The listing builds one solid part. Answer for the finished solid, in the listing's coordinates (mm). Face numbers are marked on the shaded views. A direction names the side the tool comes from. Give positions to 0.01 mm unless a question says otherwise; leave off trailing zeros. Loops run counter-clockwise (first coordinate to the right, second up) from the corner with the lowest first, then second, coordinate; pieces in that order, holes last. Notation, with made-up numbers: (59.25, 27.5) - (85.25, 27.5) arc R26 ccw to (85.25, 63.5) - close; hole circle Ø6 at (-4, 29). An arc over 180 degrees is marked (long way). Answer as CSV lines item,"result". Start each with the question number.
1) A cutting plane is placed at B-B (x = -0.75). Determine the outline of the cut face in (y, z), and give its area (3 significant figures).
2) A cutting plane is placed at C-C (y = 0). Determine the outline of the cut face in (x, z).
3) A cutting plane is placed at A-A (x = 1.5). Determine the outline of the cut face in (y, z).
4) Find the intervals of material crossed by line 1 along Z through (x, y) = (-0.75, 1.05); line 2 along Y through (x, z) = (0, 0.3); line 3 along Y through (x, z) = (11, 0.15), in increasing order.
5) For a pull along Y with two mould halves and no side action, classify the marked faces 1, 2 and 3 as pulls with the +Y half, pulls with the -Y half, needs draft (parallel to the pull), parting line crosses it, or undercut.
6) Flat-ended cylindrical pins translate along their axes: pin 1 (0.8 mm diameter, centred on x = 0.5, z = 0, fed in from +Y); pin 2 (0.8 mm diameter, centred on x = 9, z = 0, fed in from -Y). Find the tip coordinate at first contact, or state that the pin passes through.
7) A cutting plane is placed at D-D (x = 7.25). Determine the outline of the cut face in (y, z), and give its area (3 significant figures).
8) For the marked faces 4, 5, 6, 7 and 8, determine the directions among +Z, -Z, +X, -X, +Y, -Y from which every point of the face is accessible in a straight line to the end or side of a thin tool.
```python
from build123d import *

# Parameters (mm, degrees)
SALIENTE_EXTRUIR1_DEPTH = 4
SALIENTE_EXTRUIR2_DEPTH = 1.5
CROQUIS3_W              = 15
CROQUIS3_H              = 4
CORTAR_EXTRUIR1_DEPTH   = 52.086410566
CROQUIS4_R              = 1.65
CORTAR_EXTRUIR2_DEPTH   = 54.601779767
FILLET2_R               = 1
SCALE1_SCALE            = 0.3
SKETCH2_R               = 15.04592303
CUT_EXTRUDE3_DEPTH      = 0.4
SKETCH3_R               = 13.988720819
CUT_EXTRUDE4_DEPTH      = 0.4
SKETCH4_W               = 4.5
SKETCH4_H               = 0.1
BOSS_EXTRUDE1_DEPTH     = 1.6
SKETCH5_R               = 0.55
CUT_EXTRUDE5_DEPTH      = 4.4


with BuildPart() as part:
    # Sketch1 → Saliente-Extruir1 (new, symmetric)
    with BuildSketch(Plane.XY):
        with BuildLine():
            Line((-6, 0), (-6, 6))
            Line((-6, 6), (14, 6))
            Line((14, 6), (27.788799976, 17.570176974))
            ThreePointArc((27.788799976, 17.570176974), (36.898130887, 20.772215113), (30.630237093, 13.427389365))
            Line((30.630237093, 13.427389365), (17.60748156, 2.5))
            Line((17.60748156, 2.5), (35.60748156, 2.5))
            ThreePointArc((35.60748156, 2.5), (44.937608579, 0), (35.60748156, -2.5))
            Line((35.60748156, -2.5), (17.60748156, -2.5))
            Line((17.60748156, -2.5), (30.630237093, -13.427389365))
            ThreePointArc((30.630237093, -13.427389365), (36.898130887, -20.772215113), (27.788799976, -17.570176974))
            Line((27.788799976, -17.570176974), (14, -6))
            Line((14, -6), (-6, -6))
            Line((-6, -6), (-6, 0))
        make_face()
    extrude(amount=SALIENTE_EXTRUIR1_DEPTH, both=True)

    # Croquis2 → Saliente-Extruir2 (add, symmetric)
    with BuildSketch(Plane.XY):
        with BuildLine():
            Line((26.884808669, 10.284601755), (14.628097579, 0))
            Line((14.628097579, 0), (26.884808669, -10.284601755))
            ThreePointArc((26.884808669, -10.284601755), (27.660138353, -4.406075759), (31.628097579, 0))
            ThreePointArc((31.628097579, 0), (27.660138353, 4.406075759), (26.884808669, 10.284601755))
        make_face()
    extrude(amount=SALIENTE_EXTRUIR2_DEPTH, both=True)

    # Croquis3 → Cortar-Extruir1 (cut, through all)
    with BuildSketch(Plane.XY.offset(4)):
        with Locations((1.5, 0)):
            Rectangle(CROQUIS3_W, CROQUIS3_H)
    extrude(amount=-CORTAR_EXTRUIR1_DEPTH, mode=Mode.SUBTRACT)

    # Croquis4 → Cortar-Extruir2 (cut, through all)
    with BuildSketch(Plane(origin=(0, 6, 0), x_dir=(1, 0, 0), z_dir=(0, 1, 0))):
        with Locations(Location((-2.5, 0, 0), (0, 0, 180))):
            Circle(CROQUIS4_R)
    extrude(amount=-CORTAR_EXTRUIR2_DEPTH, mode=Mode.SUBTRACT)

    # Fillet2
    fillet2_edges = [part.edges().sort_by_distance(p)[0] for p in [
        (27.034037659, -6.190607199, -1.5),
        (27.034037659, 6.190607199, -1.5),
        (27.034037659, -6.190607199, 1.5),
        (27.034037659, 6.190607199, 1.5),
    ]]
    fillet(fillet2_edges, radius=FILLET2_R)


with BuildPart() as part_1:
    # Scale1: scaled about (0, 0, 0)
    add(part.part.scale(SCALE1_SCALE))

    # Sketch2 → Cut-Extrude3 (cut)
    with BuildSketch(Plane.XY.offset(1.2)):
        Circle(SKETCH2_R)
    extrude(amount=-CUT_EXTRUDE3_DEPTH, mode=Mode.SUBTRACT)

    # Sketch3 → Cut-Extrude4 (cut)
    with BuildSketch(Plane(origin=(0, 0, -1.2), x_dir=(-1, 0, 0), z_dir=(0, 0, -1))):
        Circle(SKETCH3_R)
    extrude(amount=-CUT_EXTRUDE4_DEPTH, mode=Mode.SUBTRACT)

    # Sketch4 → Boss-Extrude1 (add)
    with BuildSketch(Plane.XY.offset(0.8)):
        with Locations((0.45, -0.55)):
            Rectangle(SKETCH4_W, SKETCH4_H)
        with Locations((0.45, 0.55)):
            Rectangle(SKETCH4_W, SKETCH4_H)
    extrude(amount=-BOSS_EXTRUDE1_DEPTH)

    # Sketch5 → Cut-Extrude5 (cut)
    with BuildSketch(Plane.XZ.offset(1.8)):
        with Locations((-0.75, 0)):
            Circle(SKETCH5_R)
    extrude(amount=-CUT_EXTRUDE5_DEPTH, mode=Mode.SUBTRACT)


solid = part_1.part
```
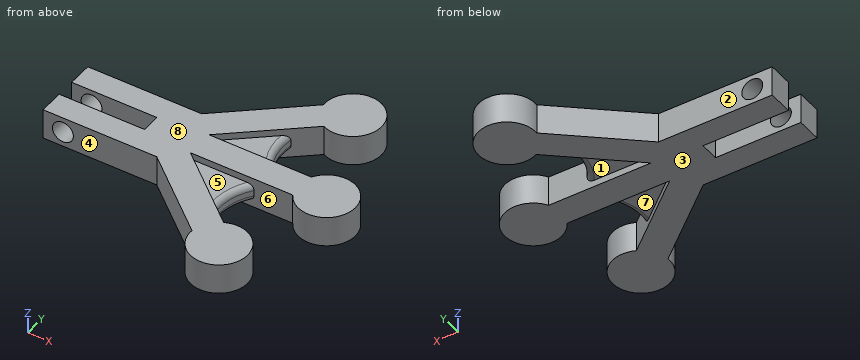
Ans:
1,outline,"(-1.8, -0.8) - (-0.5, -0.8) - (-0.5, -0.55) - (-1.8, -0.55) - close; (-1.8, 0.55) - (-0.5, 0.55) - (-0.5, 0.8) - (-1.8, 0.8) - close; (0.5, -0.8) - (1.8, -0.8) - (1.8, -0.55) - (0.5, -0.55) - close; (0.5, 0.55) - (1.8, 0.55) - (1.8, 0.8) - (0.5, 0.8) - close"
1,area,"1.30 mm2"
2,outline,"(2.7, -0.8) - (13.48, -0.8) - (13.48, 0.8) - (2.7, 0.8) - close"
3,outline,"(-1.8, -0.8) - (-0.5, -0.8) - (-0.5, 0.8) - (-1.8, 0.8) - close; (0.5, -0.8) - (1.8, -0.8) - (1.8, 0.8) - (0.5, 0.8) - close"
4,line 1,"-0.8 to -0.55, 0.55 to 0.8"
4,line 2,"-1.8 to -0.5, 0.5 to 1.8"
4,line 3,"-6.32 to -4.44, -1.13 to 1.13, 4.44 to 6.32"
5,face 1,"undercut"
5,face 2,"pulls with the +Y half"
5,face 3,"needs draft"
6,pin 1,"y = 1.8"
6,pin 2,"y = -6.82"
7,outline,"(-4.36, -0.8) - (-2.4, -0.8) - (-2.4, -0.45) - (-0.75, -0.45) - (-0.75, -0.8) - (0.75, -0.8) - (0.75, -0.45) - (2.4, -0.45) - (2.4, -0.8) - (4.36, -0.8) - (4.36, 0.8) - (2.4, 0.8) - (2.4, 0.45) - (0.75, 0.45) - (0.75, 0.8) - (-0.75, 0.8) - (-0.75, 0.45) - (-2.4, 0.45) - (-2.4, 0.8) - (-4.36, 0.8) - close"
7,area,"11.6 mm2"
8,face 4,"+Z, -Z, -X, -Y"
8,face 5,"+Z"
8,face 6,"none"
8,face 7,"-Z"
8,face 8,"+Z, +X, -X, +Y, -Y"
